For this review, take the finished solid that the model builds, in its own axes (mm). Round coordinates to 2 decimals unless told otherwise and drop trailing zeros. Order: outer loops, then holes, each group sorted by start corner. A loop starts at its lowest first (then second) coordinate and runs counter-clockwise, first axis right, second up. Notation, with made-up numbers: (54.5, 1.5) - (98.5, 1.5) arc R24 cw to (98.5, 25.5) - close; hole circle Ø4 at (17, 81). An arc over 180 degrees is marked (long way). Write each question's results on one line, items separated by ' | '. Start each with the question number.
(1) Insertion check: pin 1 Ø2 at (y, z) = (3, 2) entering from -X; pin 2 Ø1.5 at (x, y) = (2, 3) entering from -Z; pin 3 Ø1 at (y, z) = (3, -3) entering from -X; pin 4 Ø1 at (y, z) = (2, -1) entering from -X. Each pin has a flat end and moves straight along its axis. Give the tip position at first contact, or say it passes through.
(2) Take a section at A-A, the plane y = 0.7. Give the boundary of the cut face in (x, z).
(3) Take a section at D-D, the plane y = 4.5. Give the boundary of the cut face in (x, z).
(4) Take a section at B-B, the plane z = 0. Give the boundary of the cut face in (x, y), plus the area to 3 significant figures.
(5) Draft analysis for pull direction X (two halves, no side actions). For faces 1 (the flat face through (-4.318, 2.334, -0.332)), 2 (the cylindrical face through (-2, 2, 0)), 3 (the flat face through (1.871, 2.334, 3.905)), state which applies: pulls with the +X half, pulls with the -X half, needs draft (parallel to the pull), parting line crosses it, or undercut.
(6) For L1, parallel to X at y = 2.1, z = 0; L2, parallel to Z at x = -3.25, y = 3; L3, parallel to Y at x = 2.75, z = -3, list the stretches that pass through material, from the lowest coordinate up. Write a range as from..to.
(7) Take a section at C-C, the plane x = 0. Give the boundary of the cut face in (y, z).
```python
from build123d import *

# Parameters (mm, degrees)
SKETCH1_R           = 2
BOSS_EXTRUDE1_DEPTH = 5
SKETCH8_OUTSIDE_W   = 31.17
SKETCH8_OUTSIDE_H   = 32.162
SKETCH8_OUTSIDE_R   = 3.869068986
CUT_EXTRUDE1_DEPTH  = 5
CUT_EXTRUDE1_DRAFT  = -60
CHAMFER1_SIZE       = 0.2
CHAMFER2_SIZE       = 0.2


with BuildPart() as part:
    # Sketch1 → Boss-Extrude1 (new body)
    with BuildSketch(Plane(origin=(0, 0, 0), x_dir=(1, 0, 0), z_dir=(0, 1, 0))):
        Polygon((4.148216558, -2.791469037), (4.491591379, 2.196726401), (0.343374821, 4.988195438), (-4.148216558, 2.791469037), (-4.491591379, -2.196726401), (-0.343374821, -4.988195438), align=None)
        with Locations(Location((0, 0, 0), (0, 0, 270))):
            Circle(SKETCH1_R, mode=Mode.SUBTRACT)
    extrude(amount=BOSS_EXTRUDE1_DEPTH)


with BuildPart() as cut_extrude1_tool:
    # Sketch8 outside → Cut-Extrude1 (with draft: the straight prism first)
    with BuildSketch(Plane(origin=(0, 5, 0), x_dir=(1, 0, 0), z_dir=(0, 1, 0))):
        Rectangle(SKETCH8_OUTSIDE_W, SKETCH8_OUTSIDE_H)
        Circle(SKETCH8_OUTSIDE_R, mode=Mode.SUBTRACT)
    extrude(amount=-CUT_EXTRUDE1_DEPTH)
    # Cut-Extrude1: the draft: its side faces are tilted about the plane it starts from
    cut_extrude1_sides = [cut_extrude1_tool.faces().sort_by_distance(p)[0] for p in [
        (0, 2.5, 16.081),
        (15.585, 2.5, 0),
        (0, 2.5, -16.081),
        (-15.585, 2.5, 0),
        (-3.869068986, 2.5, 0),
    ]]
    draft(cut_extrude1_sides, Plane(origin=(0, 5, 0), x_dir=(1, 0, 0), z_dir=(0, 1, 0)), CUT_EXTRUDE1_DRAFT)


with BuildPart() as part_1:
    add(part.part)

    # Cut-Extrude1: cut by cut_extrude1_tool
    add(cut_extrude1_tool.part, mode=Mode.SUBTRACT)

    # Chamfer1
    chamfer1_edges = [part_1.edges().sort_by_distance(p)[0] for p in [
        (0, 5, -2),
    ]]
    chamfer(chamfer1_edges, length=CHAMFER1_SIZE)

    # Chamfer2
    chamfer2_edges = [part_1.edges().sort_by_distance(p)[0] for p in [
        (0, 0, -2),
    ]]
    chamfer(chamfer2_edges, length=CHAMFER2_SIZE)


solid = part_1.part
```
Results below:
1) pin 1: stops at x = -4.49 | pin 2: stops at z = -4.38 | pin 3: stops at x = -4.17 | pin 4: stops at x = -4.31
2) outline: (-4.49, 2.2) - (-4.15, -2.79) - (0.34, -4.99) - (4.49, -2.2) - (4.15, 2.79) - (-0.34, 4.99) - close; hole circle Ø4 at (0, 0)
3) outline: (-4.45, 1.61) - (-4.19, -2.21) arc R4.74 ccw to (-3.62, -3.05) - (-0.18, -4.73) arc R4.74 ccw to (0.83, -4.66) - (4.01, -2.52) arc R4.74 ccw to (4.45, -1.61) - (4.19, 2.21) arc R4.74 ccw to (3.62, 3.05) - (0.18, 4.73) arc R4.74 ccw to (-0.83, 4.66) - (-4.01, 2.52) arc R4.74 ccw to start; hole circle Ø4 at (0, 0)
4) outline: (-4.34, 0) - (-2.2, 0) - (-2, 0.2) - (-2, 4.8) - (-2.2, 5) - (-3.87, 5) - (-4.34, 4.73) - close; (2, 0.2) - (2.2, 0) - (4.34, 0) - (4.34, 4.73) - (3.87, 5) - (2.2, 5) - (2, 4.8) - close | area: 23.2 mm^2
5) face 1: pulls with the -X half | face 2: undercut | face 3: pulls with the +X half
6) L1: x = -4.34..-2, 2..4.34 | L2: z = -3.23..3.03 | L3: y = 0..4.88
7) outline: (0, -4.82) - (4.45, -4.82) - (5, -3.87) - (5, -2.2) - (4.8, -2) - (0.2, -2) - (0, -2.2) - close; (0, 2.2) - (0.2, 2) - (4.8, 2) - (5, 2.2) - (5, 3.87) - (4.45, 4.82) - (0, 4.82) - close
